Geometry check sheet. Reference: the model listing, model coordinates, mm. Face numbers are marked on the shaded views. A direction names the side the tool comes from. Give positions to 0.01 mm unless a question says otherwise; leave off trailing zeros. Order: outer loops, then holes, each group sorted by start corner. A loop starts at its lowest first (then second) coordinate and runs counter-clockwise, first axis right, second up.
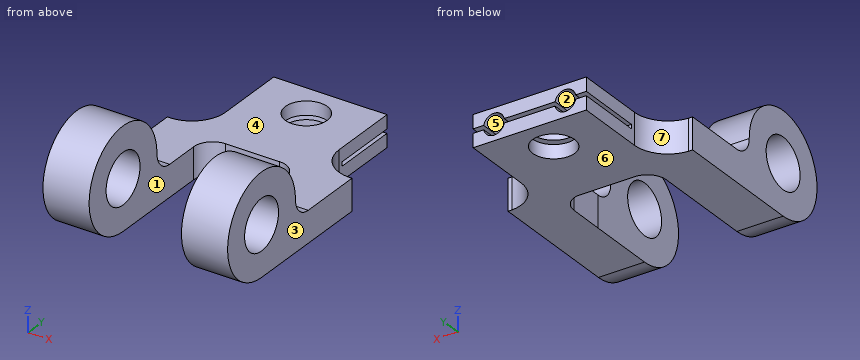
from build123d import *

# Parameters (mm, degrees)
FORK_EYE_PROFILE_R         = 12
FORK_LEG_LEFT_DEPTH        = 22
FORK_START                 = 88
SKETCH1_4_R                = 12
FORK_LEG_RIGHT_DEPTH       = 22
CLAMP_BLOCK_DEPTH          = 15
CROSS_HOLE_SKETCH_R        = 10
CROSS_HOLE_DEPTH           = 15
CLAMP_SLIT_SKETCH_W        = 2
CLAMP_SLIT_SKETCH_H        = 32
CLAMP_SLIT_DEPTH           = 137.429468957
CLAMP_SCREW_HOLES_SKETCH_R = 5
CLAMP_SCREW_HOLES_DEPTH    = 32


with BuildPart() as part:
    # Fork Eye Profile → Fork Leg Left (new body)
    with BuildSketch(Plane(origin=(0, 0, 0), x_dir=(0, 0, -1), z_dir=(1, 0, 0))):
        with BuildLine():
            Line((24, 0), (24, 64))
            Line((24, 64), (9, 64))
            Line((9, 64), (9, 33))
            ThreePointArc((9, 33), (6.363961031, 26.636038969), (0, 24))
            ThreePointArc((0, 24), (-16.970562748, -16.970562748), (24, 0))
        make_face()
        Circle(FORK_EYE_PROFILE_R, mode=Mode.SUBTRACT)
    extrude(amount=FORK_LEG_LEFT_DEPTH)



with BuildPart() as body_2:
    # Sketch1_4 → Fork Leg Right (new body)
    with BuildSketch(Plane(origin=(0, 0, 0), x_dir=(0, 0, -1), z_dir=(1, 0, 0)).offset(FORK_START)):
        with BuildLine():
            Line((24, 0), (24, 64))
            Line((24, 64), (9, 64))
            Line((9, 64), (9, 33))
            ThreePointArc((9, 33), (6.363961031, 26.636038969), (0, 24))
            ThreePointArc((0, 24), (-16.970562748, -16.970562748), (24, 0))
        make_face()
        Circle(SKETCH1_4_R, mode=Mode.SUBTRACT)
    extrude(amount=-FORK_LEG_RIGHT_DEPTH)


with BuildPart() as part_1:
    add(part.part)

    add(body_2.part)  # Clamp Block merges body 2
    # Clamp Block Profile → Clamp Block (add)
    with BuildSketch(Plane.XY.offset(-9)):
        with BuildLine():
            Line((71, 114), (17, 114))
            Line((17, 114), (17, 80))
            ThreePointArc((17, 80), (12.672648111, 69.025683194), (2.000061163, 64))
            Line((2.000061163, 64), (22, 64))
            Line((22, 64), (22, 50))
            ThreePointArc((22, 50), (24.636038969, 56.363961031), (31, 59))
            Line((31, 59), (56.929939565, 59))
            ThreePointArc((56.929939565, 59), (63.280787887, 56.377046776), (65.929863303, 50.03705013))
            Line((65.929863303, 50.03705013), (66, 33))
            Line((66, 33), (88, 33))
            Line((88, 33), (88, 64))
            ThreePointArc((88, 64), (87, 63.968719423), (86, 64))
            ThreePointArc((86, 64), (75.33809621, 69.014268273), (71, 79.968719423))
            Line((71, 79.968719423), (71, 114))
        make_face()
        with BuildLine():
            Line((22, 64), (2.000061163, 64))
            ThreePointArc((2.000061163, 64), (1.000030581, 63.968717508), (0, 64))
            Line((0, 64), (0, 59))
            Line((0, 59), (0, 33))
            Line((0, 33), (22, 33))
            Line((22, 33), (22, 50))
            Line((22, 50), (22, 64))
        make_face()
    extrude(amount=-CLAMP_BLOCK_DEPTH)

    # Cross Hole Sketch → Cross Hole (cut)
    with BuildSketch(Plane.XY.offset(-9)):
        with Locations((44, 97)):
            Circle(CROSS_HOLE_SKETCH_R)
    extrude(amount=-CROSS_HOLE_DEPTH, mode=Mode.SUBTRACT)

    # Clamp Slit Sketch → Clamp Slit (cut, through all)
    with BuildSketch(Plane.ZY.offset(-17)):
        with Locations((-16.5, 98)):
            Rectangle(CLAMP_SLIT_SKETCH_W, CLAMP_SLIT_SKETCH_H)
    extrude(amount=-CLAMP_SLIT_DEPTH, mode=Mode.SUBTRACT)

    # Clamp Screw Holes Sketch → Clamp Screw Holes (cut)
    with BuildSketch(Plane(origin=(0, 114, 0), x_dir=(1, 0, 0), z_dir=(0, 1, 0))):
        with Locations((27, 16.5)):
            Circle(CLAMP_SCREW_HOLES_SKETCH_R)
        with Locations((61, 16.5)):
            Circle(CLAMP_SCREW_HOLES_SKETCH_R)
    extrude(amount=-CLAMP_SCREW_HOLES_DEPTH, mode=Mode.SUBTRACT)


solid = part_1.part
Item 1: Set-up check for the marked faces 1, 2, 3 and 4: record each of +Z, -Z, +X, -X, +Y, -Y from which the full face is reachable in a straight line by a thin tool's end or side.
Reported:
face 1: +Z, -Z, -Y
face 2: +Y
face 3: +Z, -Z, +X, +Y, -Y
face 4: +Z, +X, -X, +Y
Item 2: Sectioned sample at B-B (y = 97). Enter the section's corners in (x, z), and give its area (3 significant figures).
Reported:
outline: (17, -24) - (34, -24) - (34, -17.5) - (31.9, -17.5) arc R5 cw to (22.1, -17.5) - (17, -17.5) - close; (17, -15.5) - (22.1, -15.5) arc R5 cw to (31.9, -15.5) - (34, -15.5) - (34, -9) - (17, -9) - close; (54, -24) - (71, -24) - (71, -17.5) - (65.9, -17.5) arc R5 cw to (56.1, -17.5) - (54, -17.5) - close; (54, -15.5) - (56.1, -15.5) arc R5 cw to (65.9, -15.5) - (71, -15.5) - (71, -9) - (54, -9) - close
area: 325 mm2
Item 3: Sectioned sample at D-D (y = 34.5). Enter the section's corners in (x, z), and give its area (3 significant figures).
Reported:
outline: (0, -24) - (22, -24) - (22, -9) - (0, -9) - close; (65.99, -24) - (88, -24) - (88, -9) - (65.99, -9) - close
area: 660 mm2
Item 4: Sectioned sample at C-C (z = -6). Enter the section's corners in (x, y), and give its area (3 significant figures).
Reported:
outline: (0, -23.24) - (22, -23.24) - (22, -10.39) - (0, -10.39) - close; (0, 10.39) - (22, 10.39) - (22, 26.29) - (0, 26.29) - close; (66, -23.24) - (88, -23.24) - (88, -10.39) - (66, -10.39) - close; (66, 10.39) - (88, 10.39) - (88, 26.29) - (66, 26.29) - close
area: 1,260 mm2
Item 5: Gauge pin test, flat ends, axial feed: pin 1 (0.6 mm diameter, centred on x = 87, z = -17.5, fed in from +Y); pin 2 (12 mm diameter, centred on x = 33, z = -12.5, fed in from -Y); pin 3 (7.5 mm diameter, centred on x = 47.5, z = -15.5, fed in from -Y). Record the tip position at first contact, or that the pin passes through.
Reported:
pin 1: stops at y = 64
pin 2: stops at y = 58.06
pin 3: stops at y = 59
Item 6: Scan lines: L1, parallel to X at y = 5, z = 21; L2, parallel to Y at x = 44.5, z = -20; L3, parallel to Y at x = 12.5, z = 0. Record each from-to range of solid material in increasing order.
Reported:
L1: x = 0 to 22, 66 to 88
L2: y = 59 to 87.01, 106.99 to 114
L3: y = -24 to -12, 12 to 24
Item 7: Draft check along X on the marked faces 5, 6 and 7. Enter one of: released by +X, released by -X, zero draft, split by the parting line, or undercut.
Reported:
face 5: undercut
face 6: zero draft
face 7: released by -X
Item 8: Sectioned sample at A-A (x = 44). Enter the section's corners in (y, z), and give its area (3 significant figures).
Reported:
outline: (59, -24) - (87, -24) - (87, -17.5) - (82, -17.5) - (82, -15.5) - (87, -15.5) - (87, -9) - (59, -9) - close; (107, -24) - (114, -24) - (114, -17.5) - (107, -17.5) - close; (107, -15.5) - (114, -15.5) - (114, -9) - (107, -9) - close
area: 501 mm2
